Part model, mm, in its own coordinate system. A direction names the side the tool comes from. Round coordinates to 2 decimals unless told otherwise and drop trailing zeros. Order: outer loops, then holes, each group sorted by start corner. A loop starts at its lowest first (then second) coordinate and runs counter-clockwise, first axis right, second up. Notation, with made-up numbers: (25.5, -24.5) - (55.5, -24.5) arc R7 ccw to (55.5, -16.5) - close; hole circle Ø6 at (87.25, 66). An arc over 180 degrees is marked (long way). Answer as a JSON object with one key per item and string values.
```python
from build123d import *

# Parameters (mm, degrees)
BOSS_EXTRUDE1_DEPTH          = 20
FILLET1_R                    = 20
FILLET2_R                    = 5
M10_TAPPED_HOLE1_D           = 8.5
M10_TAPPED_HOLE1_DEPTH       = 25
M10_TAPPED_HOLE1_CSINK_D     = 10.05
M10_TAPPED_HOLE1_CSINK_ANGLE = 90
M10_TAPPED_HOLE1_TIP         = 2.553657631


with BuildPart() as part:
    # Sketch1 → Boss-Extrude1 (new, symmetric)
    with BuildSketch(Plane.XY):
        Polygon((-41, 226), (-41, 296), (189, 296), (189, 226), (169, 226), (169, 276), (-21, 276), (-21, 226), align=None)
    extrude(amount=BOSS_EXTRUDE1_DEPTH, both=True)

    # Fillet1
    fillet1_edges = [part.edges().sort_by_distance(p)[0] for p in [
        (-21, 276, 0),
        (169, 276, 0),
        (189, 296, 0),
        (-41, 296, 0),
    ]]
    fillet(fillet1_edges, radius=FILLET1_R)

    # Fillet2
    fillet2_edges = [part.edges().sort_by_distance(p)[0] for p in [
        (-41, 251, -20),
        (74, 296, -20),
        (74, 296, 20),
        (189, 251, -20),
        (169, 241, -20),
        (74, 276, -20),
        (-35.142135624, 290.142135624, -20),
        (183.142135624, 290.142135624, -20),
        (189, 251, 20),
        (74, 276, 20),
        (169, 241, 20),
        (-21, 241, 20),
        (-35.142135624, 290.142135624, 20),
        (183.142135624, 290.142135624, 20),
        (163.142135624, 270.142135624, -20),
        (163.142135624, 270.142135624, 20),
        (-15.142135624, 270.142135624, -20),
        (-15.142135624, 270.142135624, 20),
        (-21, 241, -20),
        (-41, 251, 20),
    ]]
    fillet(fillet2_edges, radius=FILLET2_R)

    # M10 Tapped Hole1
    with Locations(Plane(origin=(-31, 226, 0), x_dir=(0, 0, -1), z_dir=(0, -1, 0))):
        with Locations((0, 0), (0, 210)):
            CounterSinkHole(M10_TAPPED_HOLE1_D / 2, M10_TAPPED_HOLE1_CSINK_D / 2, depth=M10_TAPPED_HOLE1_DEPTH, counter_sink_angle=M10_TAPPED_HOLE1_CSINK_ANGLE)
            with Locations((0, 0, -(M10_TAPPED_HOLE1_DEPTH + M10_TAPPED_HOLE1_TIP / 2))):  # 118° drill point
                Cone(0, M10_TAPPED_HOLE1_D / 2, M10_TAPPED_HOLE1_TIP, mode=Mode.SUBTRACT)


solid = part.part
```
Item 1: Cut at A-A (y = 242). Write the cut outline in (x, z).
Taken from the geometry:
{"outline": "(-41, -15) arc R5 ccw to (-36, -20) - (-26, -20) arc R5 ccw to (-21, -15) - (-21, 15) arc R5 ccw to (-26, 20) - (-36, 20) arc R5 ccw to (-41, 15) - close; (169, -15) arc R5 ccw to (174, -20) - (184, -20) arc R5 ccw to (189, -15) - (189, 15) arc R5 ccw to (184, 20) - (174, 20) arc R5 ccw to (169, 15) - close; hole circle Ø8.5 at (-31, 0); hole circle Ø8.5 at (179, 0)"}
Item 2: Probe L1, parallel to X at y = 244, z = 0; L2, parallel to Z at x = 179, y = 241; L3, parallel to X at y = 241, z = -12.5. List the from-to ranges inside material, lowest first. Write a range as from..to.
Taken from the geometry:
{"L1": "-41..-35.25, -26.75..-21, 169..174.75, 183.25..189", "L2": "-20..-4.25, 4.25..20", "L3": "-41..-21, 169..189"}
Item 3: Cut at D-D (z = -17). Write the cut outline in (x, y).
Taken from the geometry:
{"outline": "(-40.58, 226) - (-21.42, 226) - (-21.42, 256) arc R20.42 cw to (-1, 276.42) - (149, 276.42) arc R20.42 cw to (169.42, 256) - (169.42, 226) - (188.58, 226) - (188.58, 276) arc R19.58 ccw to (169, 295.58) - (-21, 295.58) arc R19.58 ccw to (-40.58, 276) - close"}
Item 4: Tool access for faces 5 (the cylindrical face through (73, 278, 19)), 6 (the flat face through (169, 241, 0)), 7 (the cylindrical face through (-33.59, 239.06, -3.37)): list every direction of +Z, -Z, +X, -X, +Y, -Y with a clear straight run to the whole face (end or side of a thin tool).
Taken from the geometry:
{"face 5": "+Z, -Y", "face 6": "+Z, -Z, -Y", "face 7": "-Y"}
Item 5: Cut at B-B (x = 118). Write the cut outline in (y, z), plus the area to 3 significant figures.
Taken from the geometry:
{"outline": "(276, -15) arc R5 ccw to (281, -20) - (291, -20) arc R5 ccw to (296, -15) - (296, 15) arc R5 ccw to (291, 20) - (281, 20) arc R5 ccw to (276, 15) - close", "area": "779 mm2"}
Item 6: Cut at C-C (z = 11.5). Write the cut outline in (x, y).
Taken from the geometry:
{"outline": "(-41, 226) - (-21, 226) - (-21, 256) arc R20 cw to (-1, 276) - (149, 276) arc R20 cw to (169, 256) - (169, 226) - (189, 226) - (189, 276) arc R20 ccw to (169, 296) - (-21, 296) arc R20 ccw to (-41, 276) - close"}
Item 7: Two-plate mould, pull along X, no slides. Class faces 1 (the flat face through (-21, 241, 0)), 2 (the cylindrical face through (73, 278, -19)), 3 (the cylindrical face through (188, 251, -18)), 4 (the cylindrical face through (-39, 251, 19)): pulls with the +X half, pulls with the -X half, needs draft (parallel to the pull), parting line crosses it, or undercut.
Taken from the geometry:
{"face 1": "undercut", "face 2": "undercut", "face 3": "pulls with the +X half", "face 4": "pulls with the -X half"}
Item 8: Drop flat-ended pins along their axis: P1, Ø5, axis at y = 283.5, z = -7, coming from the +X side; P2, Ø2, axis at y = 281, z = 12, coming from the +X side; P3, Ø24, axis at x = 55.5, z = -3, coming from the -Y side. Give the stop position or say it passes through.
Taken from the geometry:
{"P1": "x = 188.36", "P2": "x = 188.6", "P3": "y = 276"}
